Here's the drawing with two shaded views (mm, measured from the low corner). I have some questions. Round coordinates to 2 decimals unless told otherwise and drop trailing zeros. Order: outer loops, then holes, each group sorted by start corner. A loop starts at its lowest first (then second) coordinate and runs counter-clockwise, first axis right, second up.
Q1. If we section it at C-C (y = 7.75): Please give me the cut outline in (x, z), plus the area to 3 significant figures.
Q2. If I drill on line 1 (X direction, y = 4.25, z = 17.5) (1 decimal); line 2 (X direction, y = 8, z = 16); line 3 (Z direction, x = 165, y = 5), over which ranges is the centre line in solid material (lowest first)?
Q3. If we section it at B-B (z = 15): Please give me the cut outline in (x, y).
Q4. If we section it at A-A (x = 150): Please give me the cut outline in (y, z).
Q5. Will this pin go through, and if not, where does the flat tip stop? P1, Ø9.5, axis at x = 16.51, z = 15, coming from the +Y side.
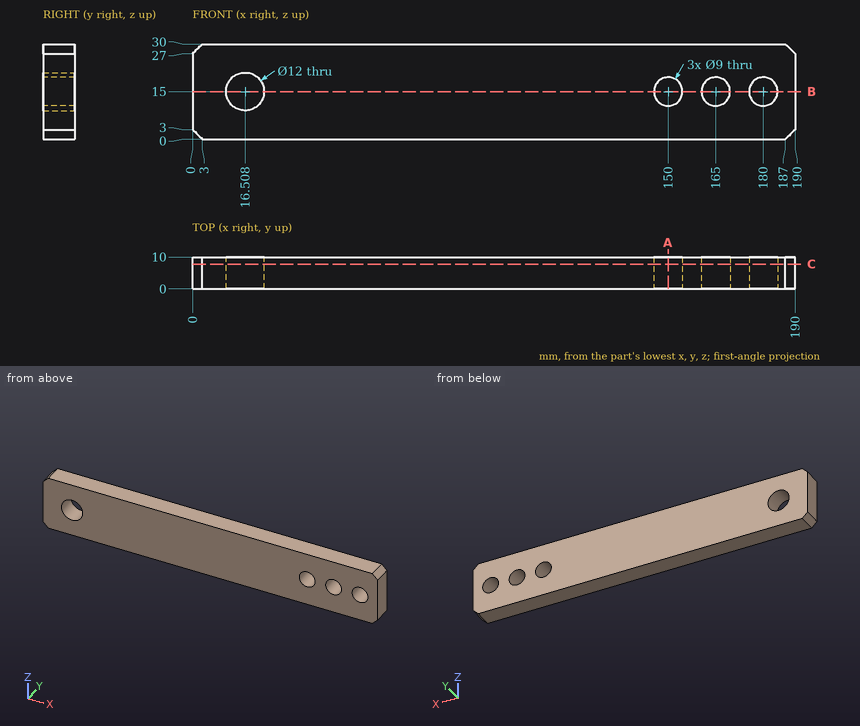
Solution:
1. outline: (0, 3) - (3, 0) - (187, 0) - (190, 3) - (190, 27) - (187, 30) - (3, 30) - (0, 27) - close; hole circle Ø12 at (16.51, 15); hole circle Ø9 at (150, 15); hole circle Ø9 at (165, 15); hole circle Ø9 at (180, 15)
1. area: 5,380 mm2
2. line 1: x = 0 to 11.1, 22 to 146.3, 153.7 to 161.3, 168.7 to 176.3, 183.7 to 190
2. line 2: x = 0 to 10.59, 22.42 to 145.61, 154.39 to 160.61, 169.39 to 175.61, 184.39 to 190
2. line 3: z = 0 to 10.5, 19.5 to 30
3. outline: (0, 0) - (10.51, 0) - (10.51, 10) - (0, 10) - close; (22.51, 0) - (145.5, 0) - (145.5, 10) - (22.51, 10) - close; (154.5, 0) - (160.5, 0) - (160.5, 10) - (154.5, 10) - close; (169.5, 0) - (175.5, 0) - (175.5, 10) - (169.5, 10) - close; (184.5, 0) - (190, 0) - (190, 10) - (184.5, 10) - close
4. outline: (0, 0) - (10, 0) - (10, 10.5) - (0, 10.5) - close; (0, 19.5) - (10, 19.5) - (10, 30) - (0, 30) - close
5. P1: passes through
